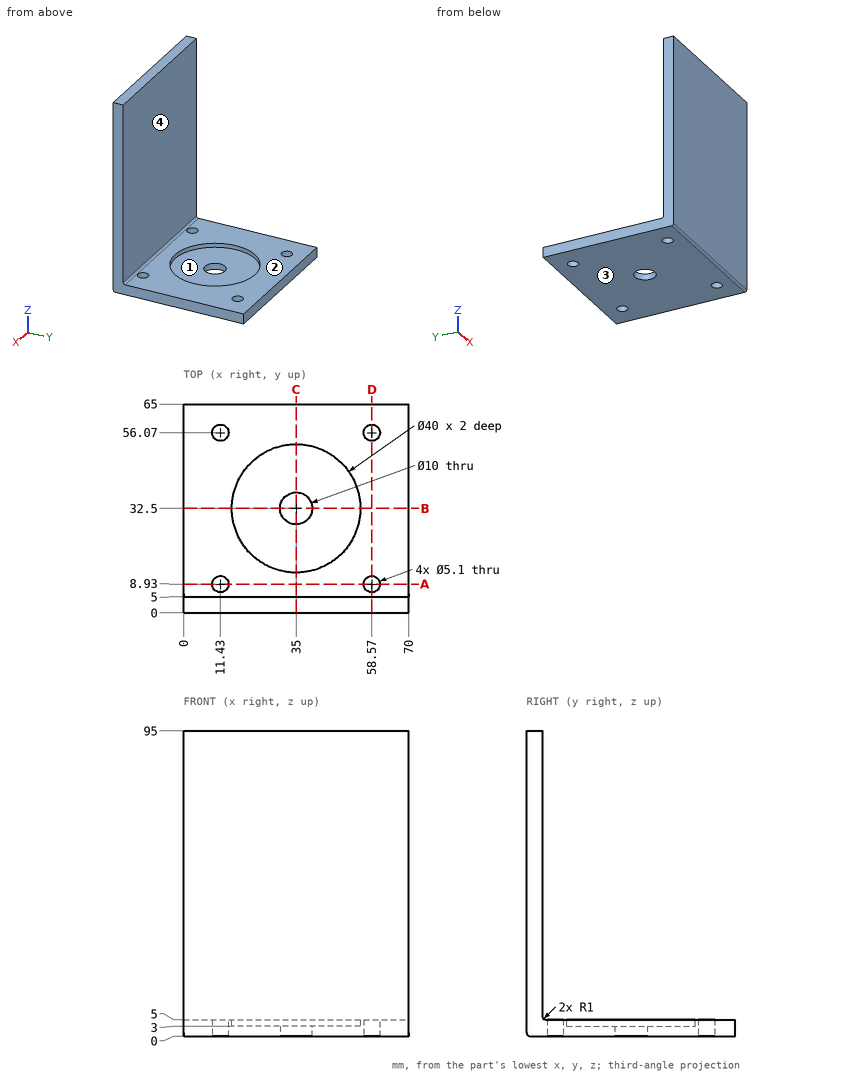
For this review, use the dimensioned drawing (mm, ordinates from the lowest corner) and the shaded views. A direction names the side the tool comes from. Coordinates: 2 decimals unless noted, no trailing zeros. Loops run counter-clockwise (first coordinate to the right, second up) from the corner with the lowest first, then second, coordinate; pieces in that order, holes last.
1. Add section B-B, the plane y = 32.5. Give the boundary of the cut face in (x, z).
2. Add section A-A, the plane y = 8.93. Give the boundary of the cut face in (x, z), then the cut area to 3 significant figures.
3. Insertion check: P1, Ø2, axis at x = 22.5, z = 21, coming from the +Y side; P2, Ø12, axis at x = 28.5, y = 42.5, coming from the +Z side; P3, Ø4, axis at x = 11.43, y = 8.93, coming from the -Z side. Each pin has a flat end and moves straight along its axis. Give the tip position at first contact, or say it passes through.
4. For the marked faces 3 and 4, list the 3-axis set-ups (+Z, -Z, +X, -X, +Y, -Y) from which the entire face can be reached by the end or side of a thin tool; tool diameter is ignored.
5. Add section D-D, the plane x = 58.57. Give the boundary of the cut face in (y, z), then the cut area to 3 significant figures.
6. For line 1 (X direction, y = 8.93, z = 3.5); line 2 (Y direction, x = 35, z = 4.3); line 3 (Y direction, x = 58.57, z = 1.65), list the stretches that pass through material, from the lowest coordinate up.
7. Add section C-C, the plane x = 35. Give the boundary of the cut face in (y, z).
8. Mouldability with a two-part tool opening along X and no side actions: class the marked faces 1 and 2 as +X half, -X half, draft (parallel to the pull), parting line (faces both ways), or undercut.
Result:
1. outline: (0, 0) - (30, 0) - (30, 3) - (15, 3) - (15, 5) - (0, 5) - close; (40, 0) - (70, 0) - (70, 5) - (55, 5) - (55, 3) - (40, 3) - close
2. outline: (0, 0) - (8.88, 0) - (8.88, 5) - (0, 5) - close; (13.98, 0) - (56.02, 0) - (56.02, 5) - (13.98, 5) - close; (61.12, 0) - (70, 0) - (70, 5) - (61.12, 5) - close
2. area: 299 mm2
3. P1: stops at y = 5
3. P2: stops at z = 3
3. P3: passes through
4. face 3: -Z, +X, -X, +Y, -Y
4. face 4: +Z, +X, -X, +Y
5. outline: (0, 1) arc R1 ccw to (1, 0) - (6.38, 0) - (6.38, 5) - (6, 5) arc R1 cw to (5, 6) - (5, 95) - (0, 95) - close; (11.48, 0) - (53.52, 0) - (53.52, 5) - (11.48, 5) - close; (58.62, 0) - (65, 0) - (65, 5) - (58.62, 5) - close
5. area: 724 mm2
6. line 1: x = 0 to 8.88, 13.98 to 56.02, 61.12 to 70
6. line 2: y = 0 to 12.5, 52.5 to 65
6. line 3: y = 0 to 6.38, 11.48 to 53.52, 58.62 to 65
7. outline: (0, 1) arc R1 ccw to (1, 0) - (27.5, 0) - (27.5, 3) - (12.5, 3) - (12.5, 5) - (6, 5) arc R1 cw to (5, 6) - (5, 95) - (0, 95) - close; (37.5, 0) - (65, 0) - (65, 5) - (52.5, 5) - (52.5, 3) - (37.5, 3) - close
8. face 1: undercut
8. face 2: draft
